Verification items for this drawing (mm, ordinates from the low corner). Round coordinates to 2 decimals unless told otherwise and drop trailing zeros. Loops run counter-clockwise (first coordinate to the right, second up) from the corner with the lowest first, then second, coordinate; pieces in that order, holes last. Notation, with made-up numbers: (35.5, 59.25) - (92.5, 59.25) arc R14 ccw to (92.5, 72.25) - close; hole circle Ø4 at (-24, 64.5). An arc over 180 degrees is marked (long way). Put each result on its own line as item: value.
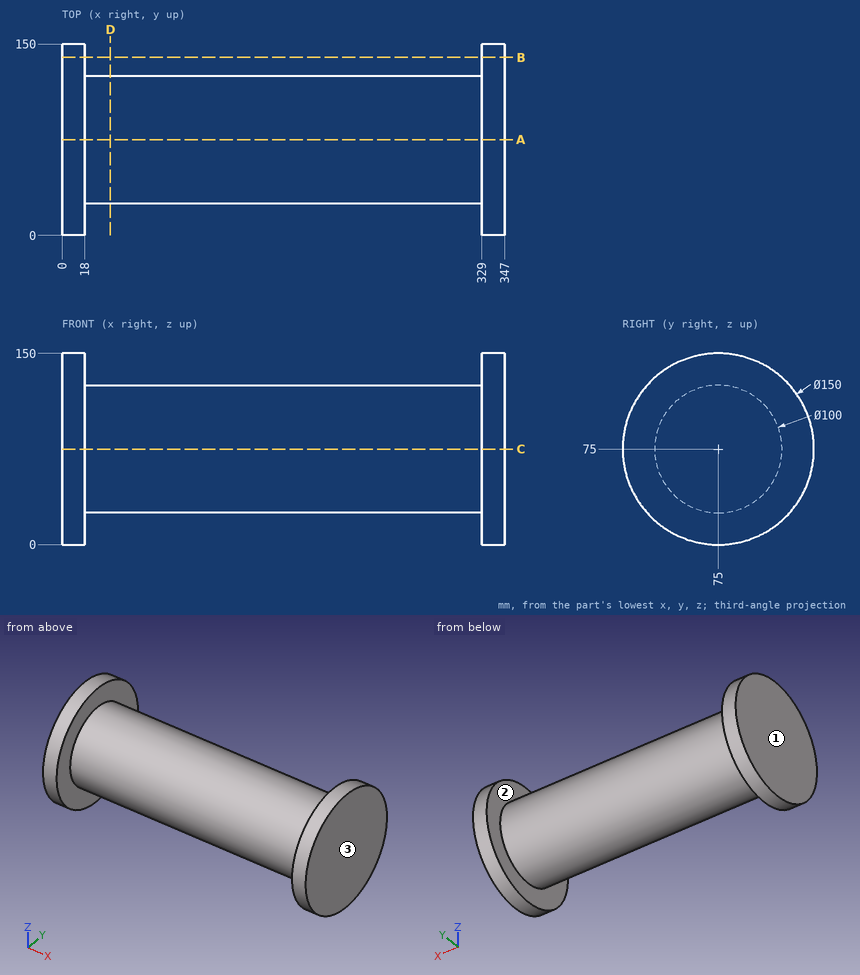
Item 1: Section check B-B on y = 139.5. Enter the section's corners in (x, z), then the cut area to 3 significant figures.
Filled sheet:
outline: (0, 36.73) - (18, 36.73) - (18, 113.27) - (0, 113.27) - close; (329, 36.73) - (347, 36.73) - (347, 113.27) - (329, 113.27) - close
area: 2,760 mm²
Item 2: Thickness scan on line 1 (X direction, y = 11.5, z = 94.5); line 2 (Y direction, x = 35, z = 77); line 3 (Z direction, x = 108, y = 76.5). Record the ranges inside material, lowest first. Write a range as from..to.
Filled sheet:
line 1: 0..18, 329..347
line 2: 25.04..124.96
line 3: 25.02..124.98
Item 3: Section check D-D on x = 38. Enter the section's corners in (y, z).
Filled sheet:
outline: circle Ø100 at (75, 75)
Item 4: Release check for a two-part mould opening along X. For the marked faces 1, 2 and 3 record: +X half, -X half, draft (parallel to the pull), parting line (faces both ways), or undercut.
Filled sheet:
face 1: -X half
face 2: undercut
face 3: +X half
Item 5: Go/stop test with flat-tipped pins: pin 1 (1.5 mm diameter, centred on x = 53, y = 66, fed in from +Z); pin 2 (12 mm diameter, centred on y = 51.5, z = 93, fed in from -X); pin 3 (10 mm diameter, centred on x = 114.5, y = 98.5, fed in from -Z); pin 4 (6 mm diameter, centred on x = 301, z = 54, fed in from -Y). Record where each tip stops, or that it passes through.
Filled sheet:
pin 1: z = 124.31
pin 2: x = 0
pin 3: z = 28.55
pin 4: y = 28.35
Item 6: Section check A-A on y = 75. Enter the section's corners in (x, z), then the cut area to 3 significant figures.
Filled sheet:
outline: (0, 0) - (18, 0) - (18, 25) - (329, 25) - (329, 0) - (347, 0) - (347, 150) - (329, 150) - (329, 125) - (18, 125) - (18, 150) - (0, 150) - close
area: 36,500 mm²
